```python
from build123d import *

# Parameters (mm, degrees)
CUT_EXTRUDE1_DEPTH = 3.82


with BuildPart() as part:
    # Sketch1 → Revolve1 (revolve)
    with BuildSketch(Plane.XY):
        with BuildLine():
            Line((0, 3), (-7.218812959, 3))
            ThreePointArc((-7.218812959, 3), (-8.195640781, 3.198737866), (-9.01716246, 3.763354074))
            Line((-9.01716246, 3.763354074), (-11.872362242, 6.72))
            Line((-11.872362242, 6.72), (-12, 6.72))
            Line((-12, 6.72), (-12, 0))
            Line((-12, 0), (0, 0))
            Line((0, 0), (0, 3))
        make_face()
    revolve(axis=Axis((0, 0, 0), (-1, 0, 0)))

    # Sketch2 → Cut-Extrude1 (cut)
    with BuildSketch(Plane.ZY.offset(12)):
        Polygon((0, 2.309401077), (-2, 1.154700538), (-2, -1.154700538), (0, -2.309401077), (2, -1.154700538), (2, 1.154700538), align=None)
    extrude(amount=-CUT_EXTRUDE1_DEPTH, mode=Mode.SUBTRACT)

    # Sketch6 → Revolve2 (revolve)
    with BuildSketch(Plane.XY, mode=Mode.PRIVATE) as revolve2_sk:
        Polygon((-9.8, 2.309401077), (-8.466666667, 0), (-7.6, 0), (-7.6, 2.309401077), align=None)
    revolve(revolve2_sk.sketch.rotate(Axis((-12, 0, 0), (1, 0, 0)), 90), axis=Axis((-12, 0, 0), (1, 0, 0)))

    # Sketch7 → Cut-Revolve2 (revolve, cut)
    with BuildSketch(Plane.XY, mode=Mode.PRIVATE) as cut_revolve2_sk:
        Polygon((-12, 2.309401077), (-12, 0), (-11.362, 0), align=None)
    revolve(cut_revolve2_sk.sketch.rotate(Axis((-12, 0, 0), (1, 0, 0)), 90), axis=Axis((-12, 0, 0), (1, 0, 0)), mode=Mode.SUBTRACT)

    # Sketch4 → Cut-Revolve1 (revolve, cut)
    with BuildSketch(Plane.XY, mode=Mode.PRIVATE) as cut_revolve1_sk:
        Polygon((-0.5, 3), (0, 2.133974596), (0.5, 3), align=None)
    revolve(cut_revolve1_sk.sketch.rotate(Axis((-0.5, 0, 0), (1, 0, 0)), 90), axis=Axis((-0.5, 0, 0), (1, 0, 0)), mode=Mode.SUBTRACT)


solid = part.part
```
Part model, mm, in its own coordinate system. A direction names the side the tool comes from. Coordinates: 2 decimals unless noted, no trailing zeros. Write each loop counter-clockwise with the first axis right and the second up, starting at its lowest first coordinate (ties: lowest second). Pieces come first, ordered by that corner, then holes.
Item 1: Probe line 1 (Y direction, x = -9.5, z = -0.25); line 2 (X direction, y = -2.5, z = -0.75); line 3 (Z direction, x = -3.75, y = 2). List the from-to ranges inside material, lowest first.
Item 2: Pin check, flat tips, straight feed: pin 1 (1.5 mm diameter, centred on x = -5.5, z = -4.5, fed in from -Y); pin 2 (3 mm diameter, centred on x = -7, y = -1, fed in from -Z); pin 3 (5 mm diameter, centred on y = -0.5, z = 0, fed in from -X); pin 4 (1 mm diameter, centred on x = -3.5, y = -3, fed in from -Z). Stop position of each tip, or through.
Item 3: Slice it at A-A (x = -2.5). Write the cut outline in (y, z), and give its area (3 significant figures).
Item 4: Mould opens along Z. For faces 4 (the face through (-12, 0, 3)), 5 (the face through (-9.196, -0.856, 3.854)), 6 (the face through (-10.827, -1.724, -1.014)) say: released by +Z, released by -Z, zero draft, split by the parting line, or undercut.
Item 5: Which spindle directions (+Z, -Z, +X, -X, +Y, -Y) get a long thin tool onto all of the face, cutting with end or side? Do faces 1 (the face through (0, 0, 0)), 2 (the face through (-11, 0, 2)), 3 (the face through (-3.91, 2.77, 1.15)). Say none if no direction does.
Results found:
1. line 1: y = -4.26 to -1.77, 1.77 to 4.26
1. line 2: x = -12 to -0.27
1. line 3: z = -2.24 to 2.24
2. pin 1: passes through
2. pin 2: stops at z = -3.27
2. pin 3: stops at x = -12
2. pin 4: stops at z = -1.66
3. outline: circle Ø6 at (0, 0)
3. area: 28.3 mm2
4. face 4: zero draft
4. face 5: split by the parting line
4. face 6: undercut
5. face 1: +Z, -Z, +X, +Y, -Y
5. face 2: -X
5. face 3: +X
